Source: CAD feature listing. Evaluate the final solid. Frame: model axes, mm. A direction names the side the tool comes from. Coordinates: 2 decimals unless noted, no trailing zeros. Order: outer loops, then holes, each group sorted by start corner. A loop starts at its lowest first (then second) coordinate and runs counter-clockwise, first axis right, second up.
```python
from build123d import *

# Parameters (mm, degrees)
BOSS_EXTRUDE1_DEPTH = 1


with BuildPart() as part:
    # Sketch1 → Boss-Extrude1 (new body)
    with BuildSketch(Plane.XY):
        with BuildLine():
            Line((1.029116593, 5.402862115), (1.029116593, 9.014895643))
            Line((1.029116593, 9.014895643), (2.817154888, 9.014895643))
            Line((2.817154888, 9.014895643), (2.817154888, 6.188993322))
            ThreePointArc((2.817154888, 6.188993322), (-0.544669265, -6.778151326), (-1.792734929, 6.559428441))
            Line((-1.792734929, 6.559428441), (-1.792734929, 9.014895643))
            Line((-1.792734929, 9.014895643), (0, 9.014895643))
            Line((0, 9.014895643), (0, 5.5))
            ThreePointArc((0, 5.5), (-0.516845415, -5.475661678), (1.029116593, 5.402862115))
        make_face()
    extrude(amount=BOSS_EXTRUDE1_DEPTH)


solid = part.part
```
1. Section query B-B, the plane x = -4.5. Output: boundary loops of the cut face in (y, z).
2. Material intervals for line 1 along X through (y, z) = (0, 0.4); line 2 along X through (y, z) = (8.25, 0.35); line 3 along Y through (x, z) = (4.25, 0.7), sorted ascending.
3. Section query D-D, the plane x = 6. Output: boundary loops of the cut face in (y, z), plus the area to 3 significant figures.
4. Contact query for flat-ended pins moving along their axis: P1, Ø0.5, axis at y = 8, z = 0.5, coming from the -X side; P2, Ø6, axis at x = -1, y = 3.5, coming from the -Z side; P3, Ø0.5, axis at y = 7, z = 0.5, coming from the +X side. Output: stop coordinate, or through.
5. Draft query along X for faces 1 (the flat face through (0, 7.3, 0.5)), 2 (the flat face through (-0.9, 9.015, 0.5)), 3 (the flat face through (2.817, 7.6, 0.5)), 4 (the flat face through (-1.793, 7.8, 0.5)). Return one class per face: +X half, -X half, draft (parallel to the pull), parting line (faces both ways), or undercut.
6. Section query A-A, the plane y = 0. Output: boundary loops of the cut face in (x, z), plus the area to 3 significant figures.
7. Section query C-C, the plane z = 0.75. Output: boundary loops of the cut face in (x, y), plus the area to 3 significant figures.
8. Access query for faces 5 (the cylindrical face through (-0.75, -5.45, 0.49)), 6 (the flat face through (1.029, 7.2, 0.5)). Directions: +Z, -Z, +X, -X, +Y, -Y. A direction counts if a zero-diameter tool reaches every point of the face in a straight line with its end or side. Return the directions, or none.
Answer key:
1. outline: (-5.1, 0) - (-3.16, 0) - (-3.16, 1) - (-5.1, 1) - close; (3.16, 0) - (5.1, 0) - (5.1, 1) - (3.16, 1) - close
2. line 1: x = -6.8 to -5.5, 5.5 to 6.8
2. line 2: x = -1.79 to 0, 1.03 to 2.82
2. line 3: y = -5.31 to -3.49, 3.49 to 5.31
3. outline: (-3.2, 0) - (3.2, 0) - (3.2, 1) - (-3.2, 1) - close
3. area: 6.40 mm2
4. P1: stops at x = -1.79
4. P2: stops at z = 0
4. P3: stops at x = 2.82
5. face 1: undercut
5. face 2: draft
5. face 3: +X half
5. face 4: -X half
6. outline: (-6.8, 0) - (-5.5, 0) - (-5.5, 1) - (-6.8, 1) - close; (5.5, 0) - (6.8, 0) - (6.8, 1) - (5.5, 1) - close
6. area: 2.60 mm2
7. outline: (-1.79, 6.56) arc R6.8 ccw (long way) to (2.82, 6.19) - (2.82, 9.01) - (1.03, 9.01) - (1.03, 5.4) arc R5.5 cw (long way) to (0, 5.5) - (0, 9.01) - (-1.79, 9.01) - close
7. area: 57.5 mm2
8. face 5: +Z, -Z
8. face 6: +Z, -Z, +Y
